Could you check a few things on this model? Use its own coordinates, in mm. A direction names the side the tool comes from. Give positions to 0.01 mm unless a question says otherwise; leave off trailing zeros. Write each loop counter-clockwise with the first axis right and the second up, starting at its lowest first coordinate (ties: lowest second). Pieces come first, ordered by that corner, then holes. Notation, with made-up numbers: M -12,-35 L 37,-35 A23 ccw 37,-23 Z; hole C 18.25,86 d1. An arc over 180 degrees is marked long. Write each question's results on one line, items separated by ' | '. Start each with the question number.
from build123d import *

# Parameters (mm, degrees)
LOWER_SHANK_SKETCH_20_R      = 10
LOWER_SHANK_20_DEPTH         = 17
GROOVE_NECK_SKETCH_16_R      = 8
GROOVE_NECK_16_DEPTH         = 3
UPPER_SHANK_SKETCH_22_R      = 11
UPPER_SHANK_22_DEPTH         = 21
HEAD_SKETCH_30_R             = 15
HEAD_30_DEPTH                = 6
SCREWDRIVER_SLOT_SKETCH_W    = 3
SCREWDRIVER_SLOT_SKETCH_H    = 32.46327366
SCREWDRIVER_SLOT_3X3_5_DEPTH = 3.5


with BuildPart() as part:
    # Lower Shank Sketch Ø20 → Lower Shank Ø20 (new body)
    with BuildSketch(Plane(origin=(0, 0, 0), x_dir=(1, 0, 0), z_dir=(0, 1, 0))):
        with Locations(Location((0, 0, 0), (0, 0, 270))):
            Circle(LOWER_SHANK_SKETCH_20_R)
    extrude(amount=LOWER_SHANK_20_DEPTH)

    # Groove Neck Sketch Ø16 → Groove Neck Ø16 (add)
    with BuildSketch(Plane(origin=(0, 17, 0), x_dir=(1, 0, 0), z_dir=(0, 1, 0))):
        with Locations(Location((0, 0, 0), (0, 0, 270))):
            Circle(GROOVE_NECK_SKETCH_16_R)
    extrude(amount=GROOVE_NECK_16_DEPTH)

    # Upper Shank Sketch Ø22 → Upper Shank Ø22 (add)
    with BuildSketch(Plane(origin=(0, 20, 0), x_dir=(1, 0, 0), z_dir=(0, 1, 0))):
        with Locations(Location((0, 0, 0), (0, 0, 90))):
            Circle(UPPER_SHANK_SKETCH_22_R)
    extrude(amount=UPPER_SHANK_22_DEPTH)

    # Head Sketch Ø30 → Head Ø30 (add)
    with BuildSketch(Plane(origin=(0, 41, 0), x_dir=(1, 0, 0), z_dir=(0, 1, 0))):
        with Locations(Location((0, 0, 0), (0, 0, 270))):
            Circle(HEAD_SKETCH_30_R)
    extrude(amount=HEAD_30_DEPTH)

    # Screwdriver Slot Sketch → Screwdriver Slot 3x3.5 (cut)
    with BuildSketch(Plane(origin=(0, 47, 0), x_dir=(1, 0, 0), z_dir=(0, 1, 0))):
        with Locations((0, -0.041354489)):
            Rectangle(SCREWDRIVER_SLOT_SKETCH_W, SCREWDRIVER_SLOT_SKETCH_H)
    extrude(amount=-SCREWDRIVER_SLOT_3X3_5_DEPTH, mode=Mode.SUBTRACT)


solid = part.part
Q1. If we section it at D-D (y = 26): Please give me the cut outline in (x, z).
Q2. If we mould it in two halves opening along Y, with no side actions, what happens to faces 5 (the face through (10, 41, -5)), 6 (the face through (-1.5, 45, 0)), 7 (the face through (-7.81, 18.48, -1.73))? For each: pulls with the +Y half, pulls with the -Y half, needs draft (parallel to the pull), parting line crosses it, or undercut.
Q3. For faces 1 (the face through (8.2, 17, 0)), 2 (the face through (10.74, 30.35, 2.38)), 3 (the face through (0, 0, 0)), 4 (the face through (1.5, 45, 0)), which set-ups out of +Z, -Z, +X, -X, +Y, -Y let a thin tool reach every point of the face, with its end or its side?
Q4. If we section it at A-A (z = 9.25): Please give me the cut outline in (x, y).
Q5. I'm going to push flat-ended pins straight in: P1, Ø8, axis at y = 35.5, z = 4, coming from the +X side; P2, Ø6, axis at y = 22.5, z = 8, coming from the -X side; P3, Ø3, axis at x = -4, y = 21, coming from the -Z side. Where does each tip first touch, or does it pass through?
Q6. If we section it at C-C (z = 0): Please give me the cut outline in (x, y).
Q7. Please list where these lines run through material, in increasing order: line 1 (Y direction, x = -8, z = 5.25); line 2 (Y direction, x = 10.5, z = 0.75); line 3 (Y direction, x = 2.75, z = -12.25). Write a range as [from, to].
Q8. If we section it at B-B (x = 0): Please give me the cut outline in (y, z), plus the area to 3 significant figures.
Determined:
1) outline: C 0,0 d22
2) face 5: pulls with the -Y half | face 6: needs draft | face 7: undercut
3) face 1: none | face 2: -Y | face 3: +Z, -Z, +X, -X, -Y | face 4: +Z, -Z, +Y
4) outline: M -11.81,41 L -5.95,41 L -5.95,20 L 5.95,20 L 5.95,41 L 11.81,41 L 11.81,47 L 1.5,47 L 1.5,43.5 L -1.5,43.5 L -1.5,47 L -11.81,47 Z; M -3.8,0 L 3.8,0 L 3.8,17 L -3.8,17 Z
5) P1: stops at x = 11 | P2: stops at x = -9.8 | P3: stops at z = -10.71
6) outline: M -15,41 L -11,41 L -11,20 L -8,20 L -8,17 L -10,17 L -10,0 L 10,0 L 10,17 L 8,17 L 8,20 L 11,20 L 11,41 L 15,41 L 15,47 L 1.5,47 L 1.5,43.5 L -1.5,43.5 L -1.5,47 L -15,47 Z
7) line 1: y = [0, 17], [20, 47] | line 2: y = [20, 47] | line 3: y = [41, 47]
8) outline: M 0,-10 L 17,-10 L 17,-8 L 20,-8 L 20,-11 L 41,-11 L 41,-15 L 43.5,-15 L 43.5,15 L 41,15 L 41,11 L 20,11 L 20,8 L 17,8 L 17,10 L 0,10 Z | area: 925 mm²
